from build123d import *

# Parameters (mm, degrees)
EXTRUDE1_DEPTH     = 12
SKETCH3_OUTSIDE_W  = 179.776
SKETCH3_OUTSIDE_H  = 179.776
SKETCH3_OUTSIDE_R  = 15
CUT_EXTRUDE1_DEPTH = 10
CUT_EXTRUDE1_DRAFT = -80
FILLET1_R          = 1


with BuildPart() as part:
    # Sketch1 → Revolve1 (revolve)
    with BuildSketch(Plane.XY, mode=Mode.PRIVATE) as revolve1_sk:
        Polygon((22, 20.955), (22, 19.476), (17, 19.476), (17, 24.5), (12, 24.5), (12, 1.5), (0, 1.5), (0, 0), (33, 0), (33, 19.476), (31.521, 20.955), align=None)
    revolve(revolve1_sk.sketch.rotate(Axis((0, 0, 0), (1, 0, 0)), 90), axis=Axis((0, 0, 0), (1, 0, 0)))

    # Sketch2 → Extrude1 (add)
    with BuildSketch(Plane.ZY):
        Polygon((0, 17.320508076), (-15, 8.660254038), (-15, -8.660254038), (0, -17.320508076), (15, -8.660254038), (15, 8.660254038), align=None)
    extrude(amount=-EXTRUDE1_DEPTH)


with BuildPart() as cut_extrude1_tool:
    # Sketch3 outside → Cut-Extrude1 (with draft: the straight prism first)
    with BuildSketch(Plane.ZY):
        Rectangle(SKETCH3_OUTSIDE_W, SKETCH3_OUTSIDE_H)
        Circle(SKETCH3_OUTSIDE_R, mode=Mode.SUBTRACT)
    extrude(amount=-CUT_EXTRUDE1_DEPTH)
    # Cut-Extrude1: the draft: its side faces are tilted about the plane it starts from
    cut_extrude1_sides = [cut_extrude1_tool.faces().sort_by_distance(p)[0] for p in [
        (5, -89.888, 0),
        (5, 0, 89.888),
        (5, 89.888, 0),
        (5, 0, -89.888),
        (5, 0, -15),
    ]]
    draft(cut_extrude1_sides, Plane.ZY, CUT_EXTRUDE1_DRAFT)


with BuildPart() as part_1:
    add(part.part)

    # Cut-Extrude1: cut by cut_extrude1_tool
    add(cut_extrude1_tool.part, mode=Mode.SUBTRACT)

    # Fillet1
    fillet1_edges = [part_1.edges().sort_by_distance(p)[0] for p in [
        (22, 0, -19.476),
        (17, 0, -19.476),
    ]]
    fillet(fillet1_edges, radius=FILLET1_R)


solid = part_1.part
Verification items for the finished model (mm, model axes). A direction names the side the tool comes from. Give positions to 0.01 mm unless a question says otherwise; leave off trailing zeros. Write each loop counter-clockwise with the first axis right and the second up, starting at its lowest first coordinate (ties: lowest second). Pieces come first, ordered by that corner, then holes. Notation, with made-up numbers: M 44.5,42.5 L 65.5,42.5 A24 ccw 65.5,54.5 Z; hole C 66.5,23 d6. An arc over 180 degrees is marked long. Write item = value, one per line.
(1) Go/stop test with flat-tipped pins: pin 1 Ø3 at (x, y) = (19, -17.5) entering from +Z; pin 2 Ø3.5 at (x, y) = (4.5, 2) entering from -Z; pin 3 Ø4 at (y, z) = (9, -4.5) entering from -X; pin 4 Ø4 at (x, z) = (7.5, -10) entering from -Y. Record where each tip stops, or that it passes through.
Found:
pin_1 = 11.1
pin_2 = -15
pin_3 = 0
pin_4 = -12.7
(2) Sectioned sample at A-A (x = 8). Record the cut outline in (y, z).
Found:
outline = M -17.32,0 L -8.66,-15 L 8.66,-15 L 17.32,0 L 8.66,15 L -8.66,15 Z
(3) Draft check along X on faces 1 (the face through (19.479, -13.163, -14.355)), 2 (the face through (5.92, 13.05, -7.4)), 3 (the face through (0.098, -7.744, -13.488)). Enter one of: released by +X, released by -X, zero draft, split by the parting line, or undercut.
Found:
face_1 = undercut
face_2 = zero draft
face_3 = released by -X
(4) Material ranges on line 1 (X direction, y = -18, z = -15.5); line 2 (X direction, y = -6, z = 18); line 3 (X direction, y = -17.5, z = 10), recorded low to high.
Found:
line_1 = 12 to 17
line_2 = 12 to 33
line_3 = 12 to 17.05, 21.95 to 32.32
(5) Access from +Z, -Z, +X, -X, +Y, -Y to the whole of each face (thin tool, end or side, straight path). Record for faces 4 (the face through (5.92, -13.05, 7.4)), 5 (the face through (22, 9.2, 18.5)), 6 (the face through (6, 0, 15)), 7 (the face through (5.916, 12.93, 7.605)), 8 (the face through (26.694, -20.777, -2.728)).
Found:
face_4 = +Z, -X, -Y
face_5 = none
face_6 = +Z, -X, +Y, -Y
face_7 = +Z, -X, +Y
face_8 = +X
(6) Sectioned sample at B-B (x = 29). Record the cut outline in (y, z) (3 decimals).
Found:
outline = C 0,0 d41.91
